Input: part model. Units: mm. Frame: model coordinates. A direction names the side the tool comes from. Coordinates: 2 decimals unless noted, no trailing zeros. Loops run counter-clockwise (first coordinate to the right, second up) from the corner with the lowest first, then second, coordinate; pieces in that order, holes last. Notation, with made-up numbers: M -5.5,12.25 L 32.5,12.25 A14 cw 32.5,35.25 Z; hole C 51,47.5 d9. An arc over 180 degrees is marked long. Use a Markdown table: item, result. Add a question column.
1. Set-up query: faces 5 (the flat face through (41, 127, 15)), 6 (the flat face through (69, 63, 30)), 7 (the flat face through (-41, 127, 15)). Return all of +Z, -Z, +X, -X, +Y, -Y with unobstructed straight access to the full face (end or side cutting, diameter ignored); none if empty.
2. Section B-B on x = 0. Output: boundary loops of the cut face in (y, z).
3. Pin query (flat end, axial travel): pin 1 (9 mm diameter, centred on y = 121.5, z = 21, fed in from +X); pin 2 (2 mm diameter, centred on x = 77, z = 29.5, fed in from -Y); pin 3 (1 mm diameter, centred on y = -49.5, z = 11, fed in from -X). Return the tip coordinate at first contact, or that it passes through.
4. Section D-D on y = 123.5. Output: boundary loops of the cut face in (x, z).
5. Line query: L1, parallel to Y at x = 0, z = 24; L2, parallel to X at y = 99, z = 6; L3, parallel to Y at x = -92, z = 22.5. Output: solid intervals per line, ascending. Write a range as [from, to].
6. Section C-C on z = 16. State how many separate pieces and enclosed holes the cut face has, then the cut area to 3 significant figures.
7. Section A-A on y = 0. Output: boundary loops of the cut face in (x, z).
8. Draft query along Y for faces 1 (the cylindrical face through (100.7, 37.88, 15.21)), 2 (the cylindrical face through (-3.69, -92.426, 31.479)), 3 (the cylindrical face through (35.83, 93.04, 15.21)), 4 (the flat face through (-1, 145, 15)). Return one class per face: +Y half, -Y half, draft (parallel to the pull), parting line (faces both ways), or undercut.
```python
from build123d import *

# Parameters (mm, degrees)
SKETCH_1_R          = 117.5
SKETCH_1_R_2        = 85
EXTRUDE_1_DEPTH     = 30
SKETCH_3_W          = 82
SKETCH_3_H          = 60
EXTRUDE_5_DEPTH     = 30
HOLE_WIZARD_M8_1_D  = 10
SKETCH_9_R          = 92.5
SKETCH_9_R_2        = 85
EXTRUDE_7_DEPTH     = 3
SKETCH_8_R          = 30
CUT_EXTRUDE_1_DEPTH = 190.526383388


with BuildPart() as part:
    # 草图1 → 凸台-拉伸1 (new body)
    with BuildSketch(Plane.XY):
        Circle(SKETCH_1_R)
        Circle(SKETCH_1_R_2, mode=Mode.SUBTRACT)
    extrude(amount=EXTRUDE_1_DEPTH)

    # 草图3 → 凸台-拉伸5 (add, through all)
    with BuildSketch(Plane.XY.offset(30)):
        with Locations((0, 115)):
            Rectangle(SKETCH_3_W, SKETCH_3_H)
    extrude(amount=-EXTRUDE_5_DEPTH)

    # M8 间隙孔1 (through all)
    with Locations(Plane(origin=(0, 0, 0), x_dir=(-1, 0, 0), z_dir=(0, 0, -1))):
        with Locations((-39.799076966, 96.083471381), (39.799076966, 96.083471381), (96.083471381, 39.799076966), (96.083471381, -39.799076966), (39.799076966, -96.083471381), (-39.799076966, -96.083471381), (-96.083471381, -39.799076966), (-96.083471381, 39.799076966)):
            Hole(HOLE_WIZARD_M8_1_D / 2)

    # 草图9 → 凸台-拉伸7 (add)
    with BuildSketch(Plane.XY.offset(30)):
        Circle(SKETCH_9_R)
        Circle(SKETCH_9_R_2, mode=Mode.SUBTRACT)
    extrude(amount=EXTRUDE_7_DEPTH)

    # 草图8 → 切除-拉伸1 (cut, through all)
    with BuildSketch(Plane(origin=(0, 0, 0), x_dir=(-1, 0, 0), z_dir=(0, 0, -1))):
        with Locations((0, 102.5)):
            Circle(SKETCH_8_R)
    extrude(amount=-CUT_EXTRUDE_1_DEPTH, mode=Mode.SUBTRACT)


solid = part.part
```
Answers below:
| question | item | result |
|---|---|---|
| 1 | face 5 | +Z, -Z, +X, +Y |
| 1 | face 6 | +Z |
| 1 | face 7 | +Z, -Z, -X, +Y |
| 2 | outline | M -117.5,0 L -85,0 L -85,33 L -92.5,33 L -92.5,30 L -117.5,30 Z; M 132.5,0 L 145,0 L 145,30 L 132.5,30 Z |
| 3 | pin 1 | stops at x = 41 |
| 3 | pin 2 | stops at y = -89.61 |
| 3 | pin 3 | stops at x = -106.8 |
| 4 | outline | M -41,0 L -21.42,0 L -21.42,30 L -41,30 Z; M 21.42,0 L 41,0 L 41,30 L 21.42,30 Z |
| 5 | L1 | y = [-117.5, -85], [132.5, 145] |
| 5 | L2 | x = [-63.29, -43.86], [-35.74, -29.8], [29.8, 35.74], [43.86, 63.29] |
| 5 | L3 | y = [-73.09, -42.68], [-36.91, 36.91], [42.68, 73.09] |
| 6 | separate pieces | 1 |
| 6 | enclosed holes | 9 |
| 6 | area | 20,100 mm² |
| 7 | outline | M -117.5,0 L -85,0 L -85,33 L -92.5,33 L -92.5,30 L -117.5,30 Z; M 85,0 L 117.5,0 L 117.5,30 L 92.5,30 L 92.5,33 L 85,33 Z |
| 8 | face 1 | undercut |
| 8 | face 2 | parting line |
| 8 | face 3 | undercut |
| 8 | face 4 | +Y half |
